```python
from build123d import *

# Parameters (mm, degrees)
SKETCH_1_R          = 60
EXTRUDE_1_DEPTH     = 80
SKETCH_2_R          = 42.5
CUT_EXTRUDE_1_DEPTH = 70
SKETCH_3_R          = 38
CUT_EXTRUDE_2_DEPTH = 70
CHAMFER_1_SIZE      = 1
SKETCH_4_R          = 52.5
SKETCH_4_R_2        = 42.5
CUT_EXTRUDE_3_DEPTH = 13
SKETCH_5_R          = 52.5
SKETCH_5_R_2        = 42.5
CUT_EXTRUDE_4_DEPTH = 13


with BuildPart() as part:
    # 草图1 → 凸台-拉伸1 (new body)
    with BuildSketch(Plane.XY):
        Circle(SKETCH_1_R)
    extrude(amount=EXTRUDE_1_DEPTH)

    # 草图2 → 切除-拉伸1 (cut)
    with BuildSketch(Plane(origin=(0, 0, 0), x_dir=(-1, 0, 0), z_dir=(0, 0, -1))):
        Circle(SKETCH_2_R)
    extrude(amount=-CUT_EXTRUDE_1_DEPTH, mode=Mode.SUBTRACT)

    # 草图3 → 切除-拉伸2 (cut)
    with BuildSketch(Plane.XY.offset(80)):
        Circle(SKETCH_3_R)
    extrude(amount=-CUT_EXTRUDE_2_DEPTH, mode=Mode.SUBTRACT)

    # 倒角1
    chamfer_1_edges = [part.edges().sort_by_distance(p)[0] for p in [
        (-60, 0, 0),
        (-60, 0, 80),
    ]]
    chamfer(chamfer_1_edges, length=CHAMFER_1_SIZE)

    # 草图4 → 切除-拉伸3 (cut)
    with BuildSketch(Plane(origin=(0, 0, 10), x_dir=(-1, 0, 0), z_dir=(0, 0, -1))):
        Circle(SKETCH_4_R)
        Circle(SKETCH_4_R_2, mode=Mode.SUBTRACT)
    extrude(amount=-CUT_EXTRUDE_3_DEPTH, mode=Mode.SUBTRACT)

    # 草图5 → 切除-拉伸4 (cut)
    with BuildSketch(Plane(origin=(0, 0, 33), x_dir=(-1, 0, 0), z_dir=(0, 0, -1))):
        Circle(SKETCH_5_R)
        Circle(SKETCH_5_R_2, mode=Mode.SUBTRACT)
    extrude(amount=-CUT_EXTRUDE_4_DEPTH, mode=Mode.SUBTRACT)


solid = part.part
```
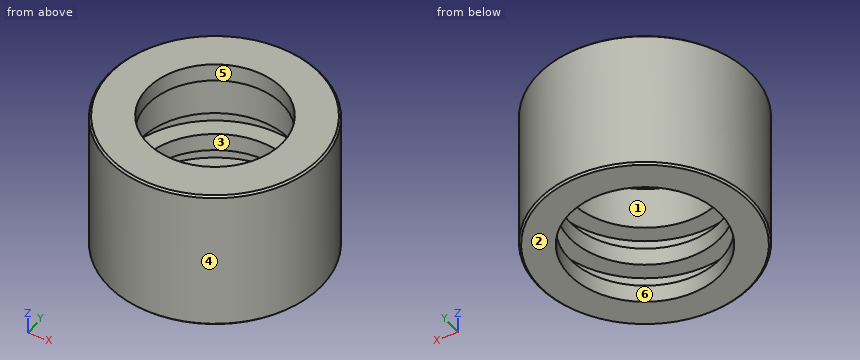
CAD build for the part. Positions are in the model's coordinates, mm. Face numbers are marked on the shaded views. A direction names the side the tool comes from. Coordinates: 2 decimals unless noted, no trailing zeros. Order: outer loops, then holes, each group sorted by start corner. A loop starts at its lowest first (then second) coordinate and runs counter-clockwise, first axis right, second up. Notation, with made-up numbers: M 88.5,-19 L 125.5,-19 A15 cw 125.5,-14 Z; hole C 22.25,66.25 d1. An arc over 180 degrees is marked long. Answer as CSV lines item,"result".
1) Drill centre lines: L1, parallel to Z at x = -28, y = 38; L2, parallel to Y at x = 0, z = 16.75; L3, parallel to Y at x = 0, z = 77. Where is each one in solid material? Low to high. Write a range as from..to.
Verdict:
L1,"0..10, 23..33, 46..80"
L2,"-60..-52.5, 52.5..60"
L3,"-60..-38, 38..60"
2) Flat gauge pins, fed straight in: P1, Ø1.5, axis at x = 10.5, z = 15.5, coming from the +Y side; P2, Ø10, axis at x = -23.5, z = 14.5, coming from the -Y side; P3, Ø2, axis at y = 22, z = 10.5, coming from the -X side (3 decimals). Where does each tip first touch, or does it go through?
Verdict:
P1,"y = 59.2"
P2,"y = -57.08"
P3,"x = -56.205"
3) Cut at C-C (z = 62). List the corners of the cut face in (x, y).
Verdict:
outline,"C 0,0 d120; hole C 0,0 d85"
4) 3-axis set-ups, long thin cutter, end or side, ignore diameter. For the marked faces 5 and 6: which of +Z, -Z, +X, -X, +Y, -Y reach the whole face in a straight line?
Verdict:
face 5,"+Z, -Z"
face 6,"-Z"
5) Cut at D-D (x = -47). Give the number of separate pieces and of enclosed holes in the cut face, then the cut area to 3 significant figures.
Verdict:
separate pieces,"1"
enclosed holes,"2"
area,"4,750 mm2"
6) Mould opens along Y. For the marked faces 1, 2, 3 and 4 say: released by +Y, released by -Y, zero draft, split by the parting line, or undercut.
Verdict:
face 1,"undercut"
face 2,"zero draft"
face 3,"undercut"
face 4,"split by the parting line"
